Model file for the job. Use its own axes, mm. Face numbers are marked on the shaded views. A direction names the side the tool comes from. Coordinates: 2 decimals unless noted, no trailing zeros. Loops run counter-clockwise (first coordinate to the right, second up) from the corner with the lowest first, then second, coordinate; pieces in that order, holes last.
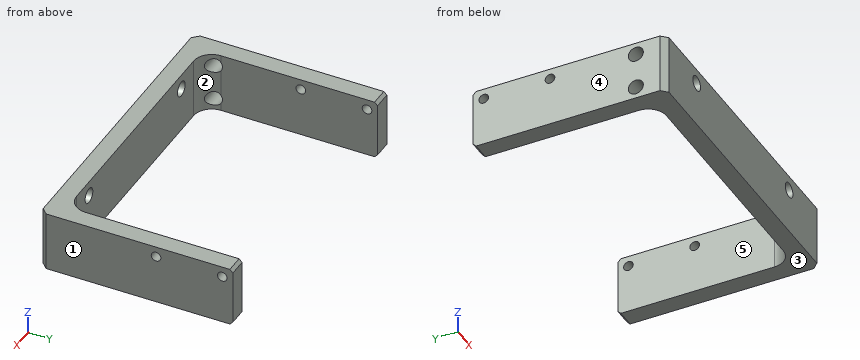
from build123d import *

# Parameters (mm, degrees)
SKETCH26_W                 = 50
SKETCH26_H                 = 32
BOSS_EXTRUDE2_DEPTH        = 5
SKETCH27_W                 = 44
SKETCH27_H                 = 29
CUT_EXTRUDE5_DEPTH         = 32.320919527
FILLET1_R                  = 3
CHAMFER1_SIZE              = 0.5
CHAMFER2_SIZE              = 1
M2_TAPPED_HOLE1_D          = 1.6
F_2_5_2_5_DIAMETER_HOLE1_D = 2.5
M3_TAPPED_HOLE2_REACH      = 54.735
M3_TAPPED_HOLE2_BORE_R     = 1.25


with BuildPart() as part:
    # Sketch26 → Boss-Extrude2 (new, symmetric)
    with BuildSketch(Plane.XY):
        Rectangle(SKETCH26_W, SKETCH26_H)
    extrude(amount=BOSS_EXTRUDE2_DEPTH, both=True)

    # Sketch27 → Cut-Extrude5 (cut, through all)
    with BuildSketch(Plane.XY.offset(5)):
        with Locations((0, 1.5)):
            Rectangle(SKETCH27_W, SKETCH27_H)
    extrude(amount=-CUT_EXTRUDE5_DEPTH, mode=Mode.SUBTRACT)

    # Fillet1
    fillet1_edges = [part.edges().sort_by_distance(p)[0] for p in [
        (22, -13, 0),
        (-22, -13, 0),
    ]]
    fillet(fillet1_edges, radius=FILLET1_R)

    # Chamfer1
    chamfer1_edges = [part.edges().sort_by_distance(p)[0] for p in [
        (-23.5, 16, -5),
        (-23.5, 16, 5),
        (23.5, 16, -5),
        (23.5, 16, 5),
    ]]
    chamfer(chamfer1_edges, length=CHAMFER1_SIZE)

    # Chamfer2
    chamfer2_edges = [part.edges().sort_by_distance(p)[0] for p in [
        (25, -16, 0),
        (-25, -16, 0),
    ]]
    chamfer(chamfer2_edges, length=CHAMFER2_SIZE)

    # M2 Tapped Hole1 (through all)
    with Locations(Plane(origin=(25, 0, 0), x_dir=(0, 0, -1), z_dir=(1, 0, 0))):
        with Locations((-3.25, 14.25), (-3.25, 3.25)):
            Hole(M2_TAPPED_HOLE1_D / 2)

    # Ø2.5 (2.5) Diameter Hole1 (through all)
    with Locations(Plane(origin=(0, -16, 0), x_dir=(-1, 0, 0), z_dir=(0, -1, 0))):
        with Locations((15, -2.5), (-15, -2.5)):
            Hole(F_2_5_2_5_DIAMETER_HOLE1_D / 2)

    # M3 Tapped Hole2 bore → M3 Tapped Hole2 (cut, up to next)
    with BuildSketch(Plane.ZY.offset(25), mode=Mode.PRIVATE) as m3_tapped_hole2_sk1:
        with Locations((-3, -11)):
            Circle(M3_TAPPED_HOLE2_BORE_R)
    m3_tapped_hole2_tool1 = extrude(m3_tapped_hole2_sk1.sketch, amount=-M3_TAPPED_HOLE2_REACH, mode=Mode.PRIVATE) & part.part
    # M3 Tapped Hole2 bore → M3 Tapped Hole2 (cut, up to next)
    with BuildSketch(Plane.ZY.offset(25), mode=Mode.PRIVATE) as m3_tapped_hole2_sk2:
        with Locations((3, -11)):
            Circle(M3_TAPPED_HOLE2_BORE_R)
    m3_tapped_hole2_tool2 = extrude(m3_tapped_hole2_sk2.sketch, amount=-M3_TAPPED_HOLE2_REACH, mode=Mode.PRIVATE) & part.part
    add(m3_tapped_hole2_tool1.solids().sort_by_distance((-25, -11, -3))[0], mode=Mode.SUBTRACT)
    add(m3_tapped_hole2_tool2.solids().sort_by_distance((-25, -11, 3))[0], mode=Mode.SUBTRACT)


solid = part.part
Q1. Slice it at D-D (x = 5.5). List the corners of the cut face in (y, z), and give its area (3 significant figures).
Answers:
outline: (-16, -5) - (-13, -5) - (-13, 5) - (-16, 5) - close
area: 30.0 mm2
Q2. Which spindle directions (+Z, -Z, +X, -X, +Y, -Y) get a long thin tool onto all of the face, cutting with end or side? Do the marked faces 4 and 5. Say none if no direction does.
Answers:
face 4: +Z, -Z, -X, +Y, -Y
face 5: +Z, -Z, +Y
Q3. Slice it at B-B (x = -15). List the corners of the cut face in (y, z), and give its area (3 significant figures).
Answers:
outline: (-16, -5) - (-13, -5) - (-13, 1.25) - (-16, 1.25) - close; (-16, 3.75) - (-13, 3.75) - (-13, 5) - (-16, 5) - close
area: 22.5 mm2
Q4. Flat gauge pins, fed straight in: P1, Ø10, axis at x = 16, y = -9, coming from the +Z side; P2, Ø1.4, axis at y = 14.25, z = 3.25, coming from the -X side; P3, Ø2, axis at y = -11, z = 3, coming from the -X side; P4, Ø6, axis at x = 7, z = -0.5, coming from the +Y side. Where does each tip first touch, or does it go through?
Answers:
P1: stops at z = 5
P2: passes through
P3: stops at x = 21.24
P4: stops at y = -13
Q5. Drill centre lines: line 1 (Y direction, x = 24, z = 3.25); line 2 (X direction, y = 13, z = -1); line 3 (Y direction, x = -23.4, z = 3.25). Where is each one in solid material? Low to high.
Answers:
line 1: y = -16 to 2.45, 4.05 to 13.45, 15.05 to 16
line 2: x = -25 to -22, 22 to 25
line 3: y = -16 to -12.22, -9.78 to 2.45, 4.05 to 13.45, 15.05 to 16
Q6. Slice it at C-C (y = -11.5). List the corners of the cut face in (x, z).
Answers:
outline: (-25, -5) - (-21.6, -5) - (-21.6, -4.15) - (-25, -4.15) - close; (-25, -1.85) - (-21.6, -1.85) - (-21.6, 1.85) - (-25, 1.85) - close; (-25, 4.15) - (-21.6, 4.15) - (-21.6, 5) - (-25, 5) - close; (21.6, -5) - (25, -5) - (25, 5) - (21.6, 5) - close
Q7. Mould opens along X. For the marked faces 1, 2 and 3 say: +X half, -X half, draft (parallel to the pull), parting line (faces both ways), or undercut.
Answers:
face 1: +X half
face 2: undercut
face 3: draft
Q8. Slice it at A-A (y = 8). List the corners of the cut face in (x, z).
Answers:
outline: (-25, -5) - (-22, -5) - (-22, 5) - (-25, 5) - close; (22, -5) - (25, -5) - (25, 5) - (22, 5) - close
